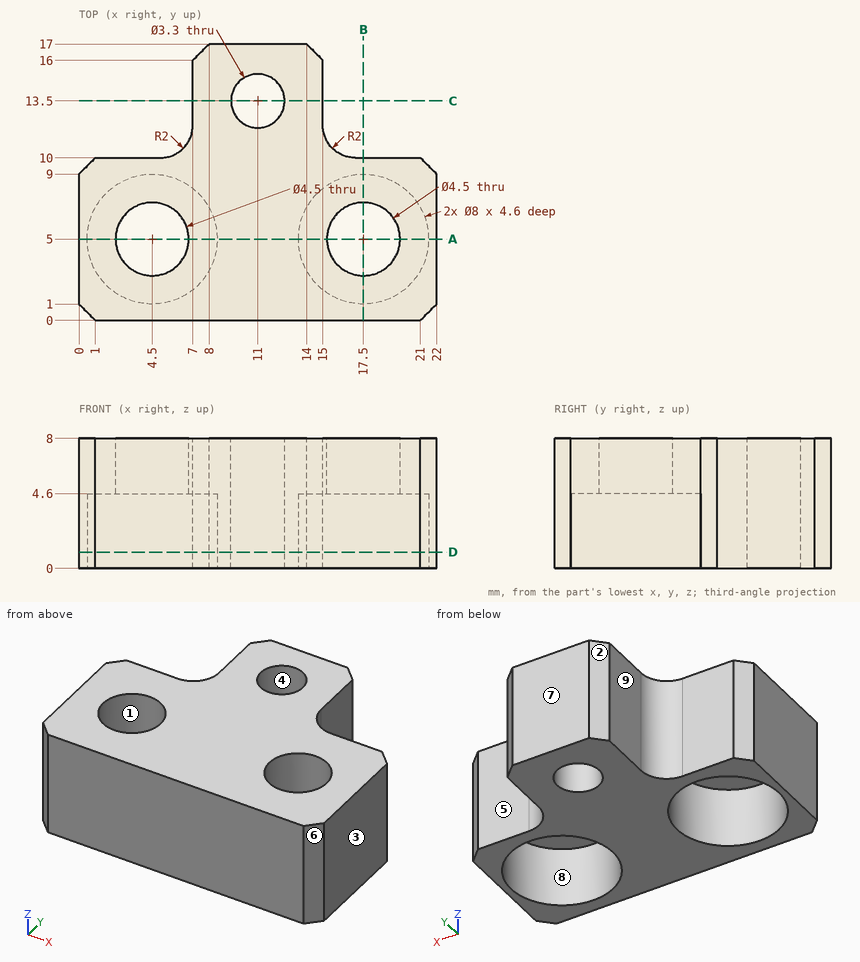
Could you check a few things on this drawing? It's one solid part, dimensions in mm from its lowest x, y, z. A direction names the side the tool comes from. Coordinates: 2 decimals unless noted, no trailing zeros. Order: outer loops, then holes, each group sorted by start corner. A loop starts at its lowest first (then second) coordinate and runs counter-clockwise, first axis right, second up.
1) We'd pull the mould along X, two halves only. Please class the marked faces 1, 2, 3 and 4: +X half, -X half, draft (parallel to the pull), parting line (faces both ways), or undercut.
2) Will these pins go through, and if not, where does the flat tip stop? pin 1 (2.5 mm diameter, centred on x = 4.5, y = 5, fed in from -Z); pin 2 (2 mm diameter, centred on x = 19, z = 4, fed in from +Y); pin 3 (1.2 mm diameter, centred on y = 13, z = 3.5, fed in from +X); pin 4 (1.2 mm diameter, centred on y = 13.5, z = 2.5, fed in from -X).
3) Which directions (+Z, -Z, +X, -X, +Y, -Y) give clear straight access to the entire face, cutting with the end or side of a thin tool? Please do the marked faces 5, 6, 7, 8 and 9.
4) Imagine slicing it at A-A on y = 5. List the corners of the cut face in (x, z) for me.
5) Imagine slicing it at C-C on y = 13.5. List the corners of the cut face in (x, z) for me, and give its area (3 significant figures).
6) Imagine slicing it at D-D on z = 1. List the corners of the cut face in (x, y) for me, and give its area (3 significant figures).
7) Imagine slicing it at B-B on x = 17.5. List the corners of the cut face in (y, z) for me.
8) I need wall thicknesses on line 1 (Y direction, x = 11, z = 3); line 2 (X direction, y = 6.75, z = 7.25); line 3 (X direction, y = 3, z = 4.5). Which ranges of each line are inside material? Lowest first, please.
Response values:
1. face 1: undercut
1. face 2: -X half
1. face 3: +X half
1. face 4: undercut
2. pin 1: passes through
2. pin 2: stops at y = 10
2. pin 3: stops at x = 15
2. pin 4: stops at x = 7
3. face 5: +Z, -Z, +X, +Y
3. face 6: +Z, -Z, +X, -Y
3. face 7: +Z, -Z, +X, -X, +Y
3. face 8: -Z
3. face 9: +Z, -Z, -X, +Y
4. outline: (0, 0) - (0.5, 0) - (0.5, 4.6) - (2.25, 4.6) - (2.25, 8) - (0, 8) - close; (6.75, 4.6) - (8.5, 4.6) - (8.5, 0) - (13.5, 0) - (13.5, 4.6) - (15.25, 4.6) - (15.25, 8) - (6.75, 8) - close; (19.75, 4.6) - (21.5, 4.6) - (21.5, 0) - (22, 0) - (22, 8) - (19.75, 8) - close
5. outline: (7, 0) - (9.35, 0) - (9.35, 8) - (7, 8) - close; (12.65, 0) - (15, 0) - (15, 8) - (12.65, 8) - close
5. area: 37.6 mm2
6. outline: (0, 1) - (1, 0) - (21, 0) - (22, 1) - (22, 9) - (21, 10) - (17, 10) arc R2 cw to (15, 12) - (15, 16) - (14, 17) - (8, 17) - (7, 16) - (7, 12) arc R2 cw to (5, 10) - (1, 10) - (0, 9) - close; hole circle Ø8 at (4.5, 5); hole circle Ø3.3 at (11, 13.5); hole circle Ø8 at (17.5, 5)
6. area: 166 mm2
7. outline: (0, 0) - (1, 0) - (1, 4.6) - (2.75, 4.6) - (2.75, 8) - (0, 8) - close; (7.25, 4.6) - (9, 4.6) - (9, 0) - (10, 0) - (10, 8) - (7.25, 8) - close
8. line 1: y = 0 to 11.85, 15.15 to 17
8. line 2: x = 0 to 3.09, 5.91 to 16.09, 18.91 to 22
8. line 3: x = 0 to 1.04, 7.96 to 14.04, 20.96 to 22
